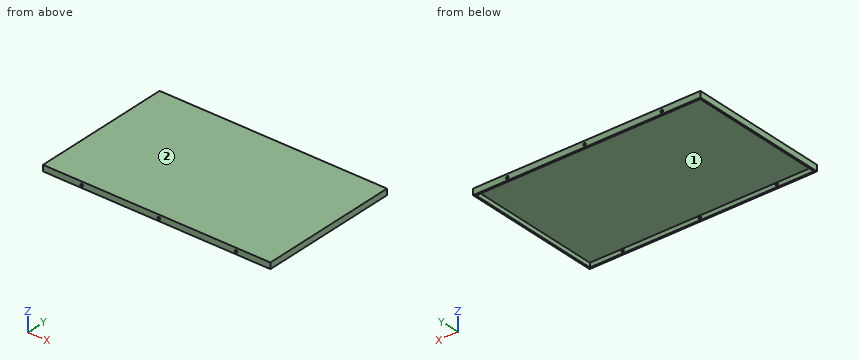
from build123d import *

# Parameters (mm, degrees)
SKETCH1_W           = 265
SKETCH1_H           = 165
BOSS_EXTRUDE1_DEPTH = 2
SKETCH2_W           = 265
SKETCH2_H           = 165
SKETCH2_W_2         = 261
SKETCH2_H_2         = 161
BOSS_EXTRUDE2_DEPTH = 5
SKETCH3_R           = 1.5
CUT_EXTRUDE1_DEPTH  = 313.209865315
LPATTERN1_COUNT     = 3
LPATTERN1_PITCH     = 90


with BuildPart() as part:
    # Sketch1 → Boss-Extrude1 (new body)
    with BuildSketch(Plane.XY):
        with Locations((132.5, 82.5)):
            Rectangle(SKETCH1_W, SKETCH1_H)
    extrude(amount=BOSS_EXTRUDE1_DEPTH)

    # Sketch2 → Boss-Extrude2 (add)
    with BuildSketch(Plane(origin=(0, 0, 0), x_dir=(-1, 0, 0), z_dir=(0, 0, -1))):
        with Locations((-132.5, 82.5)):
            Rectangle(SKETCH2_W, SKETCH2_H)
        with Locations((-132.5, 82.5)):
            Rectangle(SKETCH2_W_2, SKETCH2_H_2, mode=Mode.SUBTRACT)
    extrude(amount=BOSS_EXTRUDE2_DEPTH)

    # Sketch3 → Cut-Extrude1 (cut, through all)
    with BuildSketch(Plane(origin=(0, 165, 0), x_dir=(1, 0, 0), z_dir=(0, 1, 0))):
        with Locations(Location((225, 2, 0), (0, 0, 270))):
            Circle(SKETCH3_R)
    cut_extrude1 = extrude(amount=-CUT_EXTRUDE1_DEPTH, mode=Mode.SUBTRACT)

    # LPattern1: Cut-Extrude1 ×3
    with Locations(*[(-i * LPATTERN1_PITCH, 0, 0) for i in range(1, LPATTERN1_COUNT)]):
        add(cut_extrude1, mode=Mode.SUBTRACT)


solid = part.part
Source: CAD feature listing. Evaluate the final solid. Frame: model axes, mm. Face numbers are marked on the shaded views. Round coordinates to 2 decimals unless told otherwise and drop trailing zeros. Write each loop counter-clockwise with the first axis right and the second up, starting at its lowest first coordinate (ties: lowest second). Pieces come first, ordered by that corner, then holes. Notation, with made-up numbers: M -27,56.25 L -4,56.25 A14 cw -4,61.25 Z; hole C 53.25,50 d9. An arc over 180 degrees is marked long. One line per item, written item: value. Start each with the question number.
Item 1: Pin query (flat end, axial travel): pin 1 (1.5 mm diameter, centred on x = 108.5, y = 96.5, fed in from -Z). Return the tip coordinate at first contact, or that it passes through.
Item 2: Section query C-C (x = 197.5). Return the cut outline in (y, z).
Item 3: Section query B-B (y = 37). Return the cut outline in (x, z).
Item 4: Ray query, L1, parallel to X at y = 0.4, z = -2; L2, parallel to X at y = 127, z = -2.5; L3, parallel to Y at x = 64.5, z = -2.5. Return the intervals inside material, ascending. Write a range as from..to.
Item 5: Section query A-A (z = -2). State how many separate pieces and enclosed holes the cut face has, plus the area to 3 significant figures.
Item 6: Mould query, pull axis Y, two halves, no side actions, for the marked faces 1 and 2. Classes: pulls with the +Y half, pulls with the -Y half, needs draft (parallel to the pull), parting line crosses it, or undercut.
Result set:
1. pin 1: stops at z = 0
2. outline: M 0,-5 L 2,-5 L 2,0 L 163,0 L 163,-5 L 165,-5 L 165,2 L 0,2 Z
3. outline: M 0,-5 L 2,-5 L 2,0 L 263,0 L 263,-5 L 265,-5 L 265,2 L 0,2 Z
4. L1: x = 0..43.5, 46.5..133.5, 136.5..223.5, 226.5..265
4. L2: x = 0..2, 263..265
4. L3: y = 0..2, 163..165
5. separate pieces: 6
5. enclosed holes: 0
5. area: 1,670 mm²
6. face 1: undercut
6. face 2: needs draft
